Read the model definition and answer for the solid it produces. Units are mm, in the model's axes. A direction names the side the tool comes from. Give positions to 0.01 mm unless a question says otherwise; leave off trailing zeros. Order: outer loops, then holes, each group sorted by start corner. A loop starts at its lowest first (then second) coordinate and runs counter-clockwise, first axis right, second up. Notation, with made-up numbers: M 21.5,18 L 44.5,18 A36 cw 44.5,53 Z; hole C 67.5,-22.5 d4. An arc over 180 degrees is marked long. One line per item, written item: value.
from build123d import *

# Parameters (mm, degrees)
SKETCH1_W           = 50
SKETCH1_H           = 50
BOSS_EXTRUDE1_DEPTH = 55
SKETCH2_R           = 18.189043711
BOSS_EXTRUDE2_DEPTH = 55


with BuildPart() as part:
    # Sketch1 → Boss-Extrude1 (new body)
    with BuildSketch(Plane(origin=(0, 0, 0), x_dir=(1, 0, 0), z_dir=(0, 1, 0))):
        Rectangle(SKETCH1_W, SKETCH1_H)
    extrude(amount=BOSS_EXTRUDE1_DEPTH)

    # Sketch2 → Boss-Extrude2 (add)
    with BuildSketch(Plane.XY.offset(25)):
        with Locations((0, 27.5)):
            Circle(SKETCH2_R)
    extrude(amount=BOSS_EXTRUDE2_DEPTH)


solid = part.part
1) Consider probe 1 along Z at (x, y) = (-13.5, 4); probe 2 along Y at (x, z) = (0, 57.5); probe 3 along Y at (x, z) = (-6, 70). Determine where each line is inside the solid, lowest interval first.
Reported:
probe 1: z = -25 to 25
probe 2: y = 9.31 to 45.69
probe 3: y = 10.33 to 44.67
2) Find section A-A, the plane y = 27.5. Write down the section's boundary in (x, z).
Reported:
outline: M -25,-25 L 25,-25 L 25,25 L 18.19,25 L 18.19,80 L -18.19,80 L -18.19,25 L -25,25 Z
3) Each of these flat-tipped pins is pushed along its axis until it touches: pin 1 Ø6 at (y, z) = (14, 51.5) entering from +X; pin 2 Ø1.5 at (x, z) = (-20, 12) entering from -Y; pin 3 Ø2 at (y, z) = (7, 52) entering from +X; pin 4 Ø8 at (y, z) = (22.5, 69) entering from +X. Where does it stop, or does it pass through?
Reported:
pin 1: stops at x = 14.85
pin 2: stops at y = 0
pin 3: passes through
pin 4: stops at x = 18.16
4) Find section B-B, the plane x = 0. Write down the section's boundary in (y, z), plus the area to 3 significant figures.
Reported:
outline: M 0,-25 L 55,-25 L 55,25 L 45.69,25 L 45.69,80 L 9.31,80 L 9.31,25 L 0,25 Z
area: 4,750 mm^2
5) Find section C-C, the plane z = 41. Write down the section's boundary in (x, y), plus the area to 3 significant figures.
Reported:
outline: C 0,27.5 d36.38
area: 1,040 mm^2
6) Which of the six approach directions +Z, -Z, +X, -X, +Y, -Y give full straight-line access (tool end or side, diameter ignored) to faces 1 (the face through (0, 9, 25)), 2 (the face through (0, 27, -25))?
Reported:
face 1: +Z
face 2: -Z, +X, -X, +Y, -Y
